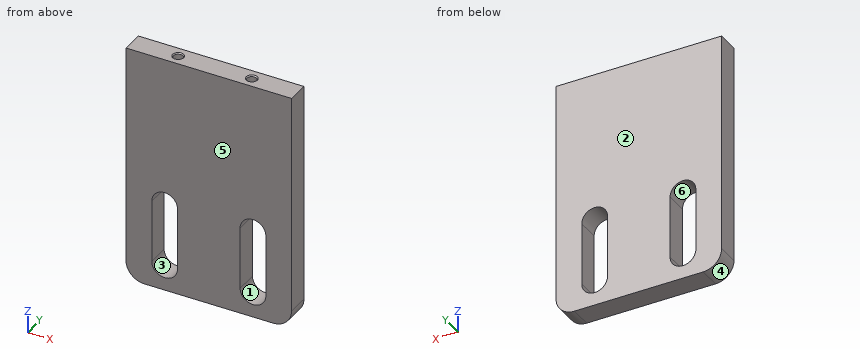
```python
from build123d import *

# Parameters (mm, degrees)
SKETCH1_W                   = 45
SKETCH1_H                   = 65
BOSS_EXTRUDE1_DEPTH         = 6
CUT_EXTRUDE1_DEPTH          = 6
FILLET2_R                   = 5
M3_TAPPED_HOLE1_D           = 2.5
M3_TAPPED_HOLE1_DEPTH       = 13.5
M3_TAPPED_HOLE1_CSINK_D     = 3.05
M3_TAPPED_HOLE1_CSINK_ANGLE = 90
M3_TAPPED_HOLE1_TIP         = 0.751075774


with BuildPart() as part:
    # Sketch1 → Boss-Extrude1 (new body)
    with BuildSketch(Plane(origin=(0, 0, 0), x_dir=(1, 0, 0), z_dir=(0, 1, 0))):
        Rectangle(SKETCH1_W, SKETCH1_H)
    extrude(amount=BOSS_EXTRUDE1_DEPTH)

    # Sketch6 → Cut-Extrude1 (cut)
    with BuildSketch(Plane(origin=(0, 6, 0), x_dir=(1, 0, 0), z_dir=(0, 1, 0))):
        with BuildLine():
            Line((-8.5, 25.5), (-8.5, 8.5))
            ThreePointArc((-8.5, 8.5), (-12, 5), (-15.5, 8.5))
            Line((-15.5, 8.5), (-15.5, 25.5))
            ThreePointArc((-15.5, 25.5), (-12, 29), (-8.5, 25.5))
        make_face()
        with BuildLine():
            Line((8.5, 25.5), (8.5, 8.5))
            ThreePointArc((8.5, 8.5), (12, 5), (15.5, 8.5))
            Line((15.5, 8.5), (15.5, 25.5))
            ThreePointArc((15.5, 25.5), (12, 29), (8.5, 25.5))
        make_face()
    extrude(amount=-CUT_EXTRUDE1_DEPTH, mode=Mode.SUBTRACT)

    # Fillet2
    fillet2_edges = [part.edges().sort_by_distance(p)[0] for p in [
        (-22.5, 3, -32.5),
        (22.5, 3, -32.5),
    ]]
    fillet(fillet2_edges, radius=FILLET2_R)

    # M3 Tapped Hole1
    with Locations(Plane.XY.offset(32.5)):
        with Locations((-10, 3), (10, 3)):
            CounterSinkHole(M3_TAPPED_HOLE1_D / 2, M3_TAPPED_HOLE1_CSINK_D / 2, depth=M3_TAPPED_HOLE1_DEPTH, counter_sink_angle=M3_TAPPED_HOLE1_CSINK_ANGLE)
            with Locations((0, 0, -(M3_TAPPED_HOLE1_DEPTH + M3_TAPPED_HOLE1_TIP / 2))):  # 118° drill point
                Cone(0, M3_TAPPED_HOLE1_D / 2, M3_TAPPED_HOLE1_TIP, mode=Mode.SUBTRACT)


solid = part.part
```
Geometry: final body of the model. Coordinates: model frame, mm. Face numbers are marked on the shaded views. A direction names the side the tool comes from. Round coordinates to 2 decimals unless told otherwise and drop trailing zeros. Order: outer loops, then holes, each group sorted by start corner. A loop starts at its lowest first (then second) coordinate and runs counter-clockwise, first axis right, second up. Notation, with made-up numbers: M 9.5,40.5 L 14.5,40.5 A30 cw 14.5,74.5 Z; hole C 31.25,-29 d5. An arc over 180 degrees is marked long. Use one line per item in the form item = value. Start each with the question number.
Q1. Material intervals for line 1 (X direction, y = 3, z = 24.5); line 2 (X direction, y = 5.55, z = -17); line 3 (Y direction, x = 10, z = 29), sorted ascending. Write a range as [from, to].
Q2. Access query for the marked faces 5 and 6. Directions: +Z, -Z, +X, -X, +Y, -Y. A direction counts if a zero-diameter tool reaches every point of the face in a straight line with its end or side. Return the directions, or none.
Q3. Cut plane B-B (y = 0.8). Return loops of the section in (x, z).
Q4. Mould query, pull axis X, two halves, no side actions, for the marked faces 1, 2, 3 and 4. Classes: +X half, -X half, draft (parallel to the pull), parting line (faces both ways), or undercut.
Q5. Cut plane C-C (x = 13). Return loops of the section in (y, z), and give its area (3 significant figures).
Q6. Cut plane A-A (z = -10). Return loops of the section in (x, y).
Geometry results:
q1.line_1 = [-22.5, -11.25], [-8.75, 8.75], [11.25, 22.5]
q1.line_2 = [-22.5, -15.5], [-8.5, 8.5], [15.5, 22.5]
q1.line_3 = [0, 1.75], [4.25, 6]
q2.face_5 = +Z, -Z, +X, -X, -Y
q2.face_6 = +Y, -Y
q3.outline = M -22.5,-27.5 A5 ccw -17.5,-32.5 L 17.5,-32.5 A5 ccw 22.5,-27.5 L 22.5,32.5 L -22.5,32.5 Z; hole M -15.5,-25.5 A3.5 ccw -8.5,-25.5 L -8.5,-8.5 A3.5 ccw -15.5,-8.5 Z; hole M 8.5,-25.5 A3.5 ccw 15.5,-25.5 L 15.5,-8.5 A3.5 ccw 8.5,-8.5 Z
q4.face_1 = undercut
q4.face_2 = draft
q4.face_3 = undercut
q4.face_4 = -X half
q5.outline = M 0,-32.5 L 6,-32.5 L 6,-28.85 L 0,-28.85 Z; M 0,-5.15 L 6,-5.15 L 6,32.5 L 0,32.5 Z
q5.area = 248 mm^2
q6.outline = M -22.5,0 L -15.5,0 L -15.5,6 L -22.5,6 Z; M -8.5,0 L 8.5,0 L 8.5,6 L -8.5,6 Z; M 15.5,0 L 22.5,0 L 22.5,6 L 15.5,6 Z
